from build123d import *

# Parameters (mm, degrees)
BASE_PLATE_SKETCH_W      = 78
BASE_PLATE_SKETCH_H      = 12
BASE_PLATE_DEPTH         = 50
UPRIGHT_BLOCK_SKETCH_W   = 42
UPRIGHT_BLOCK_SKETCH_H   = 35
UPRIGHT_BLOCK_DEPTH      = 50
BLOCK_POCKET_SKETCH_W    = 30
BLOCK_POCKET_SKETCH_H    = 22
BLOCK_POCKET_30X22_DEPTH = 79.930349043
SIDE_CUT_1_SKETCH_R      = 8
SIDE_CUT_1_DEPTH         = 10
SIDE_START               = -10
SIDE_CUT_2_SKETCH_R      = 8
SIDE_CUT_2_DEPTH         = 10
GUSSET_RIB_14MM_REACH    = 63.863
GUSSET_RIB_SKETCH_WALL_W = 175.935063468
GUSSET_RIB_SKETCH_WALL_H = 14
FRONT_PROFILE_CUT_DEPTH  = 73.429275849
RIB_START                = -20
RIB_TRIM_CUT_DEPTH       = 20


with BuildPart() as part:
    # Base Plate Sketch → Base Plate (new body)
    with BuildSketch(Plane(origin=(0, 0, 0), x_dir=(0, 0, -1), z_dir=(1, 0, 0))):
        Rectangle(BASE_PLATE_SKETCH_W, BASE_PLATE_SKETCH_H)
    extrude(amount=-BASE_PLATE_DEPTH)

    # Upright Block Sketch → Upright Block (add)
    with BuildSketch(Plane(origin=(0, 0, 0), x_dir=(0, 0, -1), z_dir=(1, 0, 0))):
        with Locations((18, 23.5)):
            Rectangle(UPRIGHT_BLOCK_SKETCH_W, UPRIGHT_BLOCK_SKETCH_H)
    extrude(amount=-UPRIGHT_BLOCK_DEPTH)

    # Block Pocket Sketch → Block Pocket 30x22 (cut, through all)
    with BuildSketch(Plane(origin=(0, 41, 0), x_dir=(1, 0, 0), z_dir=(0, 1, 0))):
        with Locations((-25, 18)):
            Rectangle(BLOCK_POCKET_SKETCH_W, BLOCK_POCKET_SKETCH_H)
    extrude(amount=-BLOCK_POCKET_30X22_DEPTH, mode=Mode.SUBTRACT)

    # Side Cut 1 Sketch → Side Cut 1 (cut)
    with BuildSketch(Plane(origin=(0, 0, 0), x_dir=(0, 0, -1), z_dir=(1, 0, 0))):
        with Locations((18, 17)):
            Circle(SIDE_CUT_1_SKETCH_R)
    extrude(amount=-SIDE_CUT_1_DEPTH, mode=Mode.SUBTRACT)

    # Side Cut 2 Sketch → Side Cut 2 (cut)
    with BuildSketch(Plane.ZY.offset(50).offset(SIDE_START)):
        with Locations(Location((-18, 17, 0), (0, 0, 180))):
            Circle(SIDE_CUT_2_SKETCH_R)
    extrude(amount=SIDE_CUT_2_DEPTH, mode=Mode.SUBTRACT)

    # Gusset Rib Sketch wall → Gusset Rib 14mm (add, up to next)
    with BuildSketch(Plane(origin=(-25, 23.5, 21), x_dir=(0, 0.697078393292, -0.716994918814), z_dir=(0, 0.716994918814, 0.697078393292)), mode=Mode.PRIVATE) as gusset_rib_14mm_sk1:
        Rectangle(GUSSET_RIB_SKETCH_WALL_W, GUSSET_RIB_SKETCH_WALL_H)
    gusset_rib_14mm_tool1 = extrude(gusset_rib_14mm_sk1.sketch, amount=-GUSSET_RIB_14MM_REACH, mode=Mode.PRIVATE) - part.part
    add(gusset_rib_14mm_tool1.solids().sort_by_distance((-25, 23.5, 21))[0])

    # Front Profile Cut Sketch → Front Profile Cut (cut, through all)
    with BuildSketch(Plane(origin=(0, 6, 0), x_dir=(1, 0, 0), z_dir=(0, 1, 0))):
        with BuildLine():
            Line((-50, -39), (-25, -39))
            ThreePointArc((-25, -39), (-42.67766953, -31.67766953), (-50, -14))
            Line((-50, -14), (-50, -39))
        make_face()
        with BuildLine():
            Line((-18, -38), (-18, -39))
            Line((-18, -39), (0, -39))
            Line((0, -39), (0, -14))
            ThreePointArc((0, -14), (-5, -29), (-18, -38))
        make_face()
    extrude(amount=-FRONT_PROFILE_CUT_DEPTH, mode=Mode.SUBTRACT)

    # Rib Trim Cut Sketch → Rib Trim Cut (cut)
    with BuildSketch(Plane.XZ.offset(6).offset(RIB_START)):
        with BuildLine():
            Line((-25, 39), (-32, 39))
            Line((-32, 39), (-32, 38))
            ThreePointArc((-32, 38), (-28.535533906, 38.748737342), (-25, 39))
        make_face()
        with BuildLine():
            ThreePointArc((-18, 38), (-21.464466094, 38.748737342), (-25, 39))
            Line((-25, 39), (-18, 39))
            Line((-18, 39), (-18, 38))
        make_face()
    extrude(amount=RIB_TRIM_CUT_DEPTH, mode=Mode.SUBTRACT)


solid = part.part
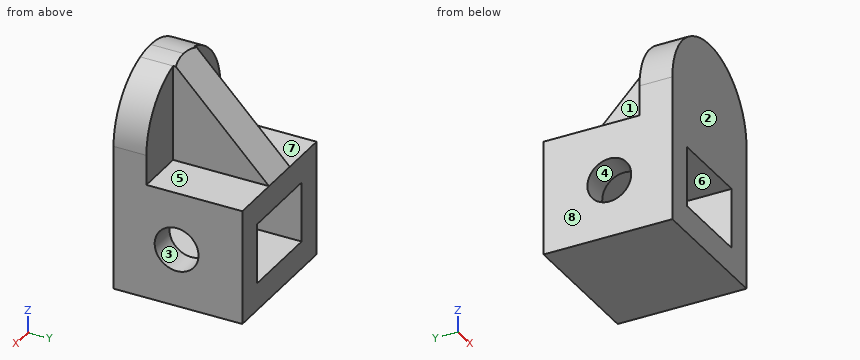
Work out the finished part from the listing and answer in its coordinate system (mm). Face numbers are marked on the shaded views. A direction names the side the tool comes from. Give positions to 0.01 mm unless a question says otherwise; leave off trailing zeros. Loops run counter-clockwise (first coordinate to the right, second up) from the corner with the lowest first, then second, coordinate; pieces in that order, holes last. Notation, with made-up numbers: (6.25, -6) - (11.25, -6) arc R31 cw to (11.25, 24) - close; hole circle Ø4 at (50.5, -9). An arc over 180 degrees is marked (long way). Answer in a Markdown table with one row per item.
(1) Section A-A (z = -18) is taken. Give the vertices of the cut face in (x, y).
Results list:
| item | result |
|---|---|
| outline | (-50, -6) - (-40, -6) - (-40, 9) - (-50, 9) - close; (-50, 25) - (-40, 25) - (-40, 41) - (-50, 41) - close; (-10, -6) - (0, -6) - (0, 9) - (-10, 9) - close; (-10, 25) - (0, 25) - (0, 41) - (-10, 41) - close |
(2) A tool of negligible diameter and unlimited length cuts with its end or side. For the marked faces 5, 6, 7 and 8, from which of +Z, -Z, +X, -X, +Y, -Y can it reach the whole face along a straight path? Write none if from no direction.
Results list:
| item | result |
|---|---|
| face 5 | +Z, +X, +Y |
| face 6 | +Y, -Y |
| face 7 | +Z, -X, +Y |
| face 8 | +Z, -Z, -X, +Y, -Y |
(3) Flat-ended cylindrical pins translate along their axes: pin 1 Ø8 at (y, z) = (34, -22.5) entering from +X; pin 2 Ø20 at (x, y) = (-38.5, 22.5) entering from +Z; pin 3 Ø9 at (x, y) = (-12.5, 17) entering from +Z; pin 4 Ø9 at (x, z) = (-39, 13.5) entering from +Y. Find the tip coordinate at first contact, or state that the pin passes through.
Results list:
| item | result |
|---|---|
| pin 1 | stops at x = 0 |
| pin 2 | stops at z = 29.85 |
| pin 3 | stops at z = 3 |
| pin 4 | stops at y = 6 |
(4) Consider L1, parallel to Z at x = -38, y = 32; L2, parallel to Y at x = -43.25, z = -18; L3, parallel to Z at x = -47, y = 17. Determine where each line is inside the solid, lowest interval first. Write a range as [from, to].
Results list:
| item | result |
|---|---|
| L1 | z = [-39, -29], [-7, 3] |
| L2 | y = [-6, 9], [25, 41] |
| L3 | z = [-39, -26], [-10, 3] |
(5) Section B-B (y = 17) is taken. Give the vertices of the cut face in (x, z), and give its area (3 significant figures).
Results list:
| item | result |
|---|---|
| outline | (-50, -39) - (0, -39) - (0, -26) - (-10, -26) - (-10, -29) - (-40, -29) - (-40, -26) - (-50, -26) - close; (-50, -10) - (-40, -10) - (-40, -7) - (-10, -7) - (-10, -10) - (0, -10) - (0, 3) - (-18, 3) - (-18, 27.69) - (-32, 27.69) - (-32, 3) - (-50, 3) - close |
| area | 1,470 mm² |
(6) Section C-C (x = -35) is taken. Give the vertices of the cut face in (y, z), and give its area (3 significant figures).
Results list:
| item | result |
|---|---|
| outline | (-6, -39) - (41, -39) - (41, -29) - (-6, -29) - close; (-6, -7) - (41, -7) - (41, 3) - (6, 3) - (6, 36.91) - (-6, 36.91) - close |
| area | 1,350 mm² |
(7) Section D-D (y = 28.5) is taken. Give the vertices of the cut face in (x, z).
Results list:
| item | result |
|---|---|
| outline | (-50, -39) - (0, -39) - (0, 3) - (-18, 3) - (-18, 15.86) - (-32, 15.86) - (-32, 3) - (-50, 3) - close; hole (-40, -29) - (-10, -29) - (-10, -7) - (-40, -7) - close |
(8) For a pull along Y with two mould halves and no side action, classify the marked faces 1, 2, 3 and 4 as pulls with the +Y half, pulls with the -Y half, needs draft (parallel to the pull), parting line crosses it, or undercut.
Results list:
| item | result |
|---|---|
| face 1 | needs draft |
| face 2 | pulls with the -Y half |
| face 3 | undercut |
| face 4 | undercut |
